from build123d import *

# Parameters (mm, degrees)
BOSS_EXTRUDE1_DEPTH = 10
CHAMFER1_SIZE       = 2


with BuildPart() as part:
    # Sketch1 → Boss-Extrude1 (new body)
    with BuildSketch(Plane.XY):
        Polygon((0, 60), (0, 0), (60, 0), (60, 2), (2, 60), align=None)
    extrude(amount=BOSS_EXTRUDE1_DEPTH)

    # Chamfer1
    chamfer1_edges = [part.edges().sort_by_distance(p)[0] for p in [
        (0, 0, 5),
    ]]
    chamfer(chamfer1_edges, length=CHAMFER1_SIZE)


solid = part.part
The listing builds one solid part. Answer for the finished solid, in the listing's coordinates (mm). Give positions to 0.01 mm unless a question says otherwise; leave off trailing zeros. Write each loop counter-clockwise with the first axis right and the second up, starting at its lowest first coordinate (ties: lowest second). Pieces come first, ordered by that corner, then holes. Notation, with made-up numbers: (-27.75, 65.25) - (29.25, 65.25) arc R6 ccw to (29.25, 71.25) - close; hole circle Ø4 at (34.5, -22). An arc over 180 degrees is marked (long way). Use a Markdown table: item, result.
1. Each of these flat-tipped pins is pushed along its axis until it touches: P1, Ø1, axis at x = 9, y = 19, coming from the -Z side; P2, Ø5, axis at x = 26.5, z = 8, coming from the +Y side; P3, Ø1.5, axis at y = 11, z = 8.5, coming from the +X side. Where does it stop, or does it pass through?
Values follow:
| item | result |
|---|---|
| P1 | stops at z = 0 |
| P2 | stops at y = 38 |
| P3 | stops at x = 51.75 |
2. Section B-B on x = 19.5 is taken. Write down the section's boundary in (y, z).
Values follow:
| item | result |
|---|---|
| outline | (0, 0) - (42.5, 0) - (42.5, 10) - (0, 10) - close |
3. Section C-C on y = 50 is taken. Write down the section's boundary in (x, z).
Values follow:
| item | result |
|---|---|
| outline | (0, 0) - (12, 0) - (12, 10) - (0, 10) - close |
4. Find the intervals of material crossed by probe 1 along X at (y, z) = (27, 7); probe 2 along X at (y, z) = (43, 6.5); probe 3 along Y at (x, z) = (28, 2), in increasing order. Write a range as from..to.
Values follow:
| item | result |
|---|---|
| probe 1 | x = 0..35 |
| probe 2 | x = 0..19 |
| probe 3 | y = 0..34 |
5. Section A-A on z = 4.75 is taken. Write down the section's boundary in (x, y).
Values follow:
| item | result |
|---|---|
| outline | (0, 2) - (2, 0) - (60, 0) - (60, 2) - (2, 60) - (0, 60) - close |
